Verification items for the finished model (mm, model axes). Face numbers are marked on the shaded views. Round coordinates to 2 decimals unless told otherwise and drop trailing zeros. Write each loop counter-clockwise with the first axis right and the second up, starting at its lowest first coordinate (ties: lowest second). Pieces come first, ordered by that corner, then holes. Notation, with made-up numbers: (27.5, -13.5) - (35.5, -13.5) arc R16 cw to (35.5, 6.5) - close; hole circle Ø2 at (49, 50.5). An arc over 180 degrees is marked (long way). Answer as a JSON object with one key per item and string values.
```python
from build123d import *


with BuildPart() as part:
    # Sketch1 → Revolve1 (revolve)
    with BuildSketch(Plane.XY, mode=Mode.PRIVATE) as revolve1_sk:
        with BuildLine():
            Line((-2.18, 0), (-2.18, 22.889528854))
            ThreePointArc((-2.18, 22.889528854), (-1.876352845, 23.999348659), (-1.05, 24.8))
            Line((-1.05, 24.8), (-0.994634547, 24.8))
            Line((-0.994634547, 24.8), (-0.994634547, 24.59))
            ThreePointArc((-0.994634547, 24.59), (-1.708849036, 23.869699743), (-1.97, 22.889528854))
            Line((-1.97, 22.889528854), (-1.97, 0))
            Line((-1.97, 0), (-2.18, 0))
        make_face()
    revolve(revolve1_sk.sketch.rotate(Axis((0, 0, 0), (0, 1, 0)), 270), axis=Axis((0, 0, 0), (0, 1, 0)))


solid = part.part
```
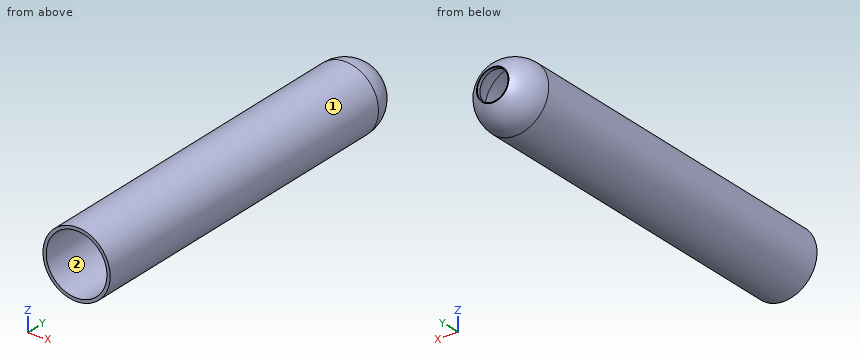
Q1. Section check A-A, the plane z = 0. Record the cut outline in (x, y).
Geometry check:
{"outline": "(-2.18, 0) - (-1.97, 0) - (-1.97, 22.89) arc R1.97 cw to (-0.99, 24.59) - (-0.99, 24.8) - (-1.05, 24.8) arc R2.18 ccw to (-2.18, 22.89) - close; (0.99, 24.59) arc R1.97 cw to (1.97, 22.89) - (1.97, 0) - (2.18, 0) - (2.18, 22.89) arc R2.18 ccw to (1.05, 24.8) - (0.99, 24.8) - close"}
Q2. Section check B-B, the plane x = 0. Record the cut outline in (y, z), then the cut area to 3 significant figures.
Geometry check:
{"outline": "(0, -2.18) - (22.89, -2.18) arc R2.18 ccw to (24.8, -1.05) - (24.8, -0.99) - (24.59, -0.99) arc R1.97 cw to (22.89, -1.97) - (0, -1.97) - close; (0, 1.97) - (22.89, 1.97) arc R1.97 cw to (24.59, 0.99) - (24.8, 0.99) - (24.8, 1.05) arc R2.18 ccw to (22.89, 2.18) - (0, 2.18) - close", "area": "10.5 mm2"}
Q3. Material ranges on line 1 along X through (y, z) = (20, -0.05); line 2 along X through (y, z) = (19.5, 1.75), recorded low to high. Write a range as [from, to].
Geometry check:
{"line 1": "x = [-2.18, -1.97], [1.97, 2.18]", "line 2": "x = [-1.3, -0.9], [0.9, 1.3]"}
Q4. Section check C-C, the plane y = 11.5. Record the cut outline in (x, z).
Geometry check:
{"outline": "circle Ø4.36 at (0, 0); hole circle Ø3.94 at (0, 0)"}
Q5. Release check for a two-part mould opening along X. For the marked faces 1 and 2 record: released by +X, released by -X, zero draft, split by the parting line, or undercut.
Geometry check:
{"face 1": "split by the parting line", "face 2": "undercut"}
Q6. Section check D-D, the plane x = -1.3. Record the cut outline in (y, z), then the cut area to 3 significant figures.
Geometry check:
{"outline": "(0, -1.75) - (22.89, -1.75) arc R1.75 ccw to (22.89, 1.75) - (0, 1.75) - (0, 1.48) - (22.89, 1.48) arc R1.48 cw to (22.89, -1.48) - (0, -1.48) - close", "area": "13.7 mm2"}
